from build123d import *

# Parameters (mm, degrees)
SKETCH1_R            = 19.5
BOSS_EXTRUDE1_DEPTH  = 16
M8_TAPPED_HOLE1_D    = 6.8
LPATTERN1_COUNT      = 2
LPATTERN1_PITCH      = 300
LPATTERN1_COUNT_DIR2 = 2
LPATTERN1_PITCH_DIR2 = 44


with BuildPart() as part:
    # Sketch1 → Boss-Extrude1 (new, symmetric)
    with BuildSketch(Plane.XY):
        Polygon((1050, 100), (1006.698729811, 125), (-1006.698729811, 125), (-1050, 100), (-1050, -100), (-1006.698729811, -125), (1006.698729811, -125), (1050, -100), align=None)
        with Locations((-390, 80)):
            Circle(SKETCH1_R, mode=Mode.SUBTRACT)
        with Locations((-90, 80)):
            Circle(SKETCH1_R, mode=Mode.SUBTRACT)
        with Locations(Location((-90, -80, 0), (0, 0, 180))):
            Circle(SKETCH1_R, mode=Mode.SUBTRACT)
        with Locations(Location((-390, -80, 0), (0, 0, 180))):
            Circle(SKETCH1_R, mode=Mode.SUBTRACT)
        with Locations((390, -80)):
            Circle(SKETCH1_R, mode=Mode.SUBTRACT)
        with Locations((90, -80)):
            Circle(SKETCH1_R, mode=Mode.SUBTRACT)
        with Locations(Location((90, 80, 0), (0, 0, 180))):
            Circle(SKETCH1_R, mode=Mode.SUBTRACT)
        with Locations(Location((390, 80, 0), (0, 0, 180))):
            Circle(SKETCH1_R, mode=Mode.SUBTRACT)
    extrude(amount=BOSS_EXTRUDE1_DEPTH, both=True)

    # M8 Tapped Hole1 (through all)
    with Locations(Plane.XY.offset(16)):
        with Locations((640, 22)):
            m8_tapped_hole1 = Hole(M8_TAPPED_HOLE1_D / 2)

    # LPattern1: M8 Tapped Hole1 2 × 2
    with Locations(*[(i * LPATTERN1_PITCH, -j * LPATTERN1_PITCH_DIR2, 0) for i in range(LPATTERN1_COUNT) for j in range(LPATTERN1_COUNT_DIR2) if (i, j) != (0, 0)]):
        add(m8_tapped_hole1, mode=Mode.SUBTRACT)


solid = part.part
Check sheet for the modelled part. Datum: model origin and axes. Units: mm. Give positions to 0.01 mm unless a question says otherwise; leave off trailing zeros. Order: outer loops, then holes, each group sorted by start corner. A loop starts at its lowest first (then second) coordinate and runs counter-clockwise, first axis right, second up. Notation, with made-up numbers: (-34.5, 72.25) - (24.5, 72.25) arc R19 cw to (24.5, 108.25) - close; hole circle Ø3 at (5.25, 17.25). An arc over 180 degrees is marked (long way). Answer as CSV lines item,"result".
1. Section check A-A (x = 90). Record the boundary of the cut face in (y, z).
Result sheet:
outline,"(-125, -16) - (-99.5, -16) - (-99.5, 16) - (-125, 16) - close; (-60.5, -16) - (60.5, -16) - (60.5, 16) - (-60.5, 16) - close; (99.5, -16) - (125, -16) - (125, 16) - (99.5, 16) - close"
2. Section check B-B (z = -1.5). State how many separate pieces and enclosed holes the cut face has, then the cut area to 3 significant figures.
Result sheet:
separate pieces,"1"
enclosed holes,"12"
area,"513,000 mm²"
3. Mould release check, pull along Y, two halves, no side actions. Record for faces 1 (the face through (-85.773, -60.964, -0.224)), 2 (the face through (-15, 2, -16)), 3 (the face through (-14, -125, 0)): released by +Y, released by -Y, zero draft, split by the parting line, or undercut.
Result sheet:
face 1,"undercut"
face 2,"zero draft"
face 3,"released by -Y"
4. Section check C-C (y = -80). Record the boundary of the cut face in (x, z).
Result sheet:
outline,"(-1050, -16) - (-409.5, -16) - (-409.5, 16) - (-1050, 16) - close; (-370.5, -16) - (-109.5, -16) - (-109.5, 16) - (-370.5, 16) - close; (-70.5, -16) - (70.5, -16) - (70.5, 16) - (-70.5, 16) - close; (109.5, -16) - (370.5, -16) - (370.5, 16) - (109.5, 16) - close; (409.5, -16) - (1050, -16) - (1050, 16) - (409.5, 16) - close"
5. Scan lines: probe 1 along Y at (x, z) = (940, -3.5); probe 2 along Y at (x, z) = (-90, -6.5); probe 3 along X at (y, z) = (98, 8). Record each from-to range of solid material in increasing order. Write a range as from..to.
Result sheet:
probe 1,"-125..-25.4, -18.6..18.6, 25.4..125"
probe 2,"-125..-99.5, -60.5..60.5, 99.5..125"
probe 3,"-1050..-397.5, -382.5..-97.5, -82.5..82.5, 97.5..382.5, 397.5..1050"
